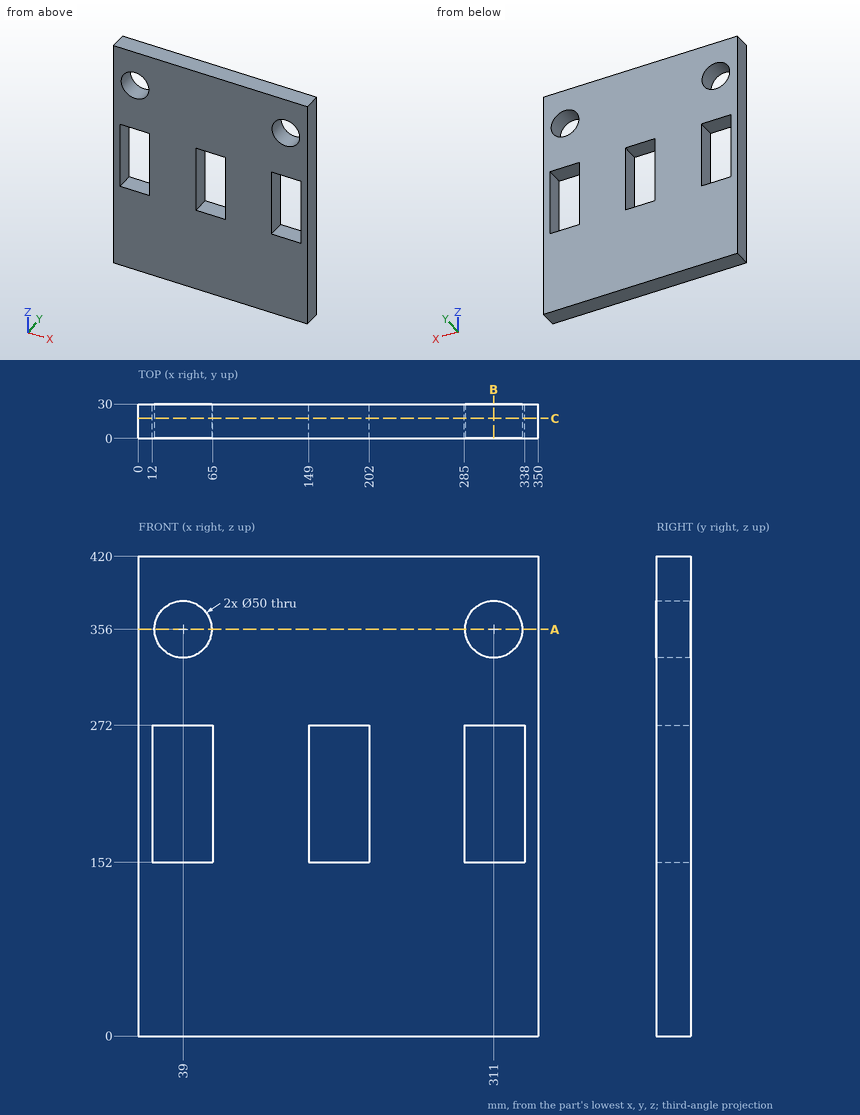
Check sheet for the drawn part. Datum: minimum x, y, z corner. Units: mm. Give positions to 0.01 mm unless a question says otherwise; leave off trailing zeros. Order: outer loops, then holes, each group sorted by start corner. A loop starts at its lowest first (then second) coordinate and runs counter-clockwise, first axis right, second up. Notation, with made-up numbers: (12, -16) - (22, -16) arc R20 cw to (22, 10) - close; hole circle Ø1 at (-1, 72.5). An arc over 180 degrees is marked (long way). Write item = value, one per line. Start each with the question number.
1) Section check B-B (x = 311). Enter the section's corners in (y, z), then the cut area to 3 significant figures.
2) Scan lines: L1, parallel to X at y = 23.75, z = 356; L2, parallel to X at y = 21.5, z = 183; L3, parallel to Z at x = 319, y = 4.75. Record each from-to range of solid material in increasing order.
3) Section check A-A (z = 356). Enter the section's corners in (x, y).
4) Section check C-C (y = 17.5). Enter the section's corners in (x, z).
Geometry check:
q1.outline = (0, 0) - (30, 0) - (30, 152) - (0, 152) - close; (0, 272) - (30, 272) - (30, 331) - (0, 331) - close; (0, 381) - (30, 381) - (30, 420) - (0, 420) - close
q1.area = 7,500 mm2
q2.L1 = 0 to 14, 64 to 286, 336 to 350
q2.L2 = 0 to 12, 65 to 149, 202 to 285, 338 to 350
q2.L3 = 0 to 152, 272 to 332.31, 379.69 to 420
q3.outline = (0, 0) - (14, 0) - (14, 30) - (0, 30) - close; (64, 0) - (286, 0) - (286, 30) - (64, 30) - close; (336, 0) - (350, 0) - (350, 30) - (336, 30) - close
q4.outline = (0, 0) - (350, 0) - (350, 420) - (0, 420) - close; hole (12, 152) - (65, 152) - (65, 272) - (12, 272) - close; hole circle Ø50 at (39, 356); hole (149, 152) - (202, 152) - (202, 272) - (149, 272) - close; hole (285, 152) - (338, 152) - (338, 272) - (285, 272) - close; hole circle Ø50 at (311, 356)
